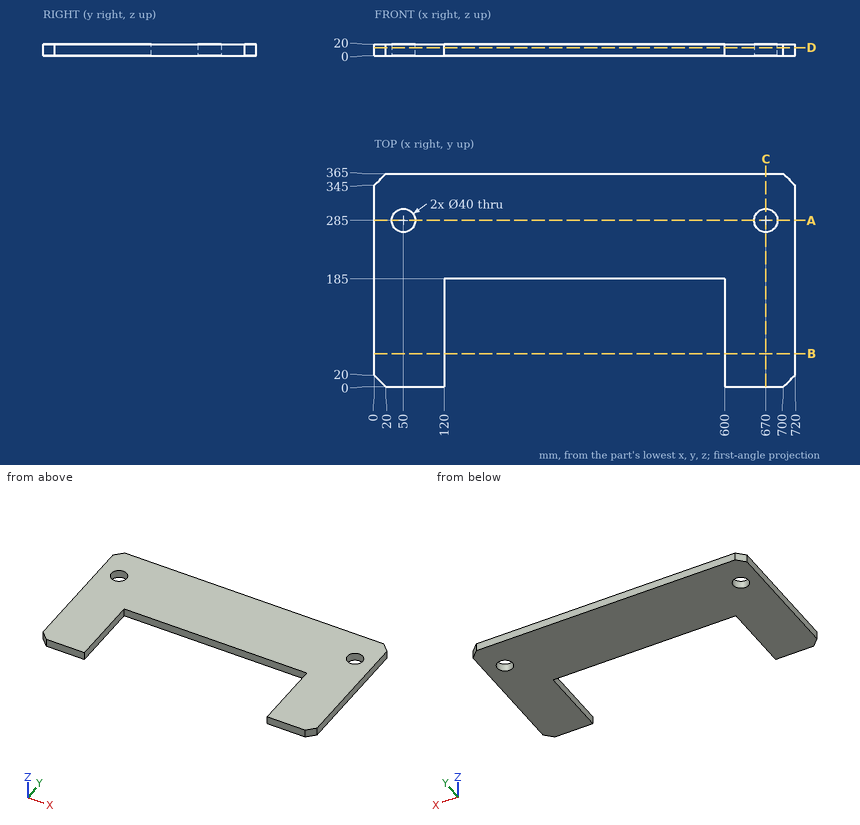
Study the drawing (mm; zero at the part's minimum x, y, z) and answer. Coordinates: 2 decimals unless noted, no trailing zeros. Loops run counter-clockwise (first coordinate to the right, second up) from the corner with the lowest first, then second, coordinate; pieces in that order, holes last. Notation, with made-up numbers: (54, 58) -> (70, 58) arc R27 ccw to (70, 91) -> close; hole circle Ø2 at (-30.75, 5.25). An arc over 180 degrees is marked (long way). Write item = value, one per line. Start each with the question number.
1) Given P1, Ø10, axis at x = 339, z = 10.5, coming from the -Y side; P2, Ø24, axis at x = 670, y = 285, coming from the +Z side (3 decimals), each flat-ended and moving along its own axis, determine where each tip first touches the part or whether it passes through.
2) The part is cut by section B-B, the plane y = 57. Determine the outline of the cut face in (x, z), plus the area to 3 significant figures.
3) The part is cut by section D-D, the plane z = 13.75. Determine the outline of the cut face in (x, y).
4) Find the intervals of material crossed by L1, parallel to Y at x = 670, z = 4; L2, parallel to X at y = 51, z = 12; L3, parallel to X at y = 285, z = 4.25, in increasing order. Write a range as from..to.
5) The part is cut by section C-C, the plane x = 670. Determine the outline of the cut face in (y, z), plus the area to 3 significant figures.
6) The part is cut by section A-A, the plane y = 285. Determine the outline of the cut face in (x, z), plus the area to 3 significant figures.
Result:
q1.P1 = 185
q1.P2 = through
q2.outline = (0, 0) -> (120, 0) -> (120, 20) -> (0, 20) -> close; (600, 0) -> (720, 0) -> (720, 20) -> (600, 20) -> close
q2.area = 4,800 mm²
q3.outline = (0, 20) -> (20, 0) -> (120, 0) -> (120, 185) -> (600, 185) -> (600, 0) -> (700, 0) -> (720, 20) -> (720, 345) -> (700, 365) -> (20, 365) -> (0, 345) -> close; hole circle Ø40 at (50, 285); hole circle Ø40 at (670, 285)
q4.L1 = 0..265, 305..365
q4.L2 = 0..120, 600..720
q4.L3 = 0..30, 70..650, 690..720
q5.outline = (0, 0) -> (265, 0) -> (265, 20) -> (0, 20) -> close; (305, 0) -> (365, 0) -> (365, 20) -> (305, 20) -> close
q5.area = 6,500 mm²
q6.outline = (0, 0) -> (30, 0) -> (30, 20) -> (0, 20) -> close; (70, 0) -> (650, 0) -> (650, 20) -> (70, 20) -> close; (690, 0) -> (720, 0) -> (720, 20) -> (690, 20) -> close
q6.area = 12,800 mm²
